```python
from build123d import *

# Parameters (mm, degrees)
BOSS_EXTRUDE1_DEPTH     = 20
F_3_4_10_TAPPED_HOLE1_D = 16.66748


with BuildPart() as part:
    # Sketch1 → Boss-Extrude1 (new body)
    with BuildSketch(Plane.XY):
        Polygon((0, 195), (5, 200), (165, 200), (170, 195), (170, 0), (0, 0), align=None)
    extrude(amount=BOSS_EXTRUDE1_DEPTH)

    # 3/4-10 Tapped Hole1 (through all)
    with Locations(Plane(origin=(85, 155, 20), x_dir=(1, 0, 0), z_dir=(0, 0, 1))):
        with Locations((0, 0)):
            Hole(F_3_4_10_TAPPED_HOLE1_D / 2)


solid = part.part
```
The listing builds one solid part. Answer for the finished solid, in the listing's coordinates (mm). Coordinates: 2 decimals unless noted, no trailing zeros. Write each loop counter-clockwise with the first axis right and the second up, starting at its lowest first coordinate (ties: lowest second). Pieces come first, ordered by that corner, then holes. Notation, with made-up numbers: (7, 79) - (44, 79) arc R28 ccw to (44, 108) - close; hole circle Ø4 at (-13, 2). An arc over 180 degrees is marked (long way). Return JSON: item names as keys, results as strings. Group by question number.
1. A cutting plane is placed at A-A, the plane x = 85. Determine the outline of the cut face in (y, z).
2. A cutting plane is placed at B-B, the plane y = 155. Determine the outline of the cut face in (x, z).
3. Determine the mould class of faces 1 (the cylindrical face through (91.142, 160.632, 9.86)), 2 (the flat face through (0, 96, 10)), 3 (the flat face through (84, 200, 10)) for opening direction Y: released by +Y, released by -Y, zero draft, split by the parting line, or undercut.
4. Straight lines are drawn through the part: L1, parallel to Y at x = 85, z = 9; L2, parallel to Y at x = 91.5, z = 1.75. For each, find the intervals that lie inside material, in ascending order.
Ans:
{
 "1": {"outline": "(0, 0) - (146.67, 0) - (146.67, 20) - (0, 20) - close; (163.33, 0) - (200, 0) - (200, 20) - (163.33, 20) - close"},
 "2": {"outline": "(0, 0) - (76.67, 0) - (76.67, 20) - (0, 20) - close; (93.33, 0) - (170, 0) - (170, 20) - (93.33, 20) - close"},
 "3": {"face 1": "undercut", "face 2": "zero draft", "face 3": "released by +Y"},
 "4": {"L1": "0 to 146.67, 163.33 to 200", "L2": "0 to 149.78, 160.22 to 200"}
}
